Model file for the job. Use its own axes, mm. Round coordinates to 2 decimals unless told otherwise and drop trailing zeros. Write each loop counter-clockwise with the first axis right and the second up, starting at its lowest first coordinate (ties: lowest second). Pieces come first, ordered by that corner, then holes.
```python
from build123d import *

# Parameters (mm, degrees)
SKETCH1_W           = 400
SKETCH1_H           = 120
BOSS_EXTRUDE1_DEPTH = 5
CUT_EXTRUDE1_DEPTH  = 209.865985742


with BuildPart() as part:
    # Sketch1 → Boss-Extrude1 (new body)
    with BuildSketch(Plane.XY):
        Rectangle(SKETCH1_W, SKETCH1_H)
    extrude(amount=BOSS_EXTRUDE1_DEPTH)

    # Sketch2 → Cut-Extrude1 (cut, through all)
    with BuildSketch(Plane.XY.offset(5)):
        with BuildLine():
            Line((-147, 0), (-147, -96.926835552))
            ThreePointArc((-147, -96.926835552), (-160, -109.926835552), (-173, -96.926835552))
            Line((-173, -96.926835552), (-173, 0))
            ThreePointArc((-173, 0), (-160, 13), (-147, 0))
        make_face()
        with BuildLine():
            Line((147, 0), (147, -96.926835552))
            ThreePointArc((147, -96.926835552), (160, -109.926835552), (173, -96.926835552))
            Line((173, -96.926835552), (173, 0))
            ThreePointArc((173, 0), (160, 13), (147, 0))
        make_face()
    extrude(amount=-CUT_EXTRUDE1_DEPTH, mode=Mode.SUBTRACT)


solid = part.part
```
1) Cut at C-C on x = -160. List the corners of the cut face in (y, z).
2) Pull direction X, two halves, no side cores. Call faces 1 (the face through (-3, 1, 5)), 2 (the face through (160, 13, 3)): released by +X, released by -X, zero draft, split by the parting line, or undercut.
3) Cut at A-A on y = -15. List the corners of the cut face in (x, z).
4) Cut at B-B on z = 1.85. List the corners of the cut face in (x, y), and give its area (3 significant figures).
5) Wall check: probe 1 along X at (y, z) = (-49.5, 4.5); probe 2 along X at (y, z) = (11.5, 3.1); probe 3 along Y at (x, z) = (-169, 0.95). Give the ranges that are in metal, low to high.
6) Flat gauge pin, fed straight in: pin 1 Ø1 at (x, y) = (-103, -44.5) entering from -Z. Where does the tip first touch, or does it go through?
Result sheet:
1. outline: (13, 0) - (60, 0) - (60, 5) - (13, 5) - close
2. face 1: zero draft
2. face 2: undercut
3. outline: (-200, 0) - (-173, 0) - (-173, 5) - (-200, 5) - close; (-147, 0) - (147, 0) - (147, 5) - (-147, 5) - close; (173, 0) - (200, 0) - (200, 5) - (173, 5) - close
4. outline: (-200, -60) - (-173, -60) - (-173, 0) arc R13 cw to (-147, 0) - (-147, -60) - (147, -60) - (147, 0) arc R13 cw to (173, 0) - (173, -60) - (200, -60) - (200, 60) - (-200, 60) - close
4. area: 44,300 mm2
5. probe 1: x = -200 to -173, -147 to 147, 173 to 200
5. probe 2: x = -200 to -166.06, -153.94 to 153.94, 166.06 to 200
5. probe 3: y = 9.38 to 60
6. pin 1: stops at z = 0
